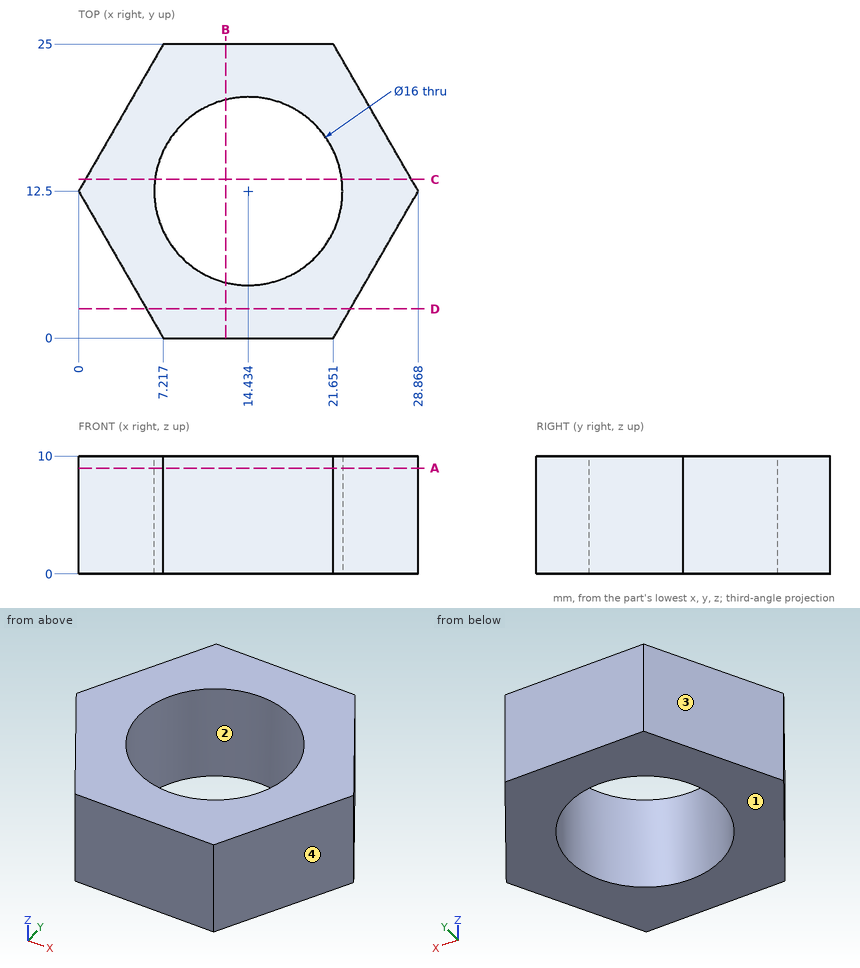
Here's the drawing with two shaded views (mm, measured from the low corner). I have some questions. Coordinates: 2 decimals unless noted, no trailing zeros. Order: outer loops, then holes, each group sorted by start corner. A loop starts at its lowest first (then second) coordinate and runs counter-clockwise, first axis right, second up.
Item 1: If we section it at D-D, the plane y = 2.5: List the corners of the cut face in (x, z) for me, then the cut area to 3 significant figures.
Response values:
outline: (5.77, 0) - (23.09, 0) - (23.09, 10) - (5.77, 10) - close
area: 173 mm2
Item 2: I'm going to push flat-ended pins straight in: pin 1 Ø1 at (x, z) = (6, 5.5) entering from -Y; pin 2 Ø1 at (x, z) = (4.5, 6) entering from +Y; pin 3 Ø1 at (x, z) = (6.5, 2) entering from -Y (1 decimal). Where does each tip first touch, or does it pass through?
Response values:
pin 1: stops at y = 1.24
pin 2: stops at y = 21.16
pin 3: stops at y = 0.4
Item 3: If we section it at A-A, the plane z = 9: List the corners of the cut face in (x, y) for me, then the cut area to 3 significant figures.
Response values:
outline: (0, 12.5) - (7.22, 0) - (21.65, 0) - (28.87, 12.5) - (21.65, 25) - (7.22, 25) - close; hole circle Ø16 at (14.43, 12.5)
area: 340 mm2
Item 4: Thinking about a two-plate mould opening in X: for the marked faces 1, 2, 3 and 4, which applies, pulls with the +X half, pulls with the -X half, needs draft (parallel to the pull), parting line crosses it, or undercut?
Response values:
face 1: needs draft
face 2: undercut
face 3: pulls with the -X half
face 4: pulls with the +X half
Item 5: If we section it at C-C, the plane y = 13.5: List the corners of the cut face in (x, z) for me, then the cut area to 3 significant figures.
Response values:
outline: (0.58, 0) - (6.5, 0) - (6.5, 10) - (0.58, 10) - close; (22.37, 0) - (28.29, 0) - (28.29, 10) - (22.37, 10) - close
area: 118 mm2
Item 6: If we section it at B-B, the plane x = 12.5: List the corners of the cut face in (y, z) for me.
Response values:
outline: (0, 0) - (4.74, 0) - (4.74, 10) - (0, 10) - close; (20.26, 0) - (25, 0) - (25, 10) - (20.26, 10) - close
Item 7: I need wall thicknesses on probe 1 along Y at (x, z) = (10, 3.25); probe 2 along X at (y, z) = (19.5, 5.5) (1 decimal); probe 3 along Y at (x, z) = (7.5, 1.25). Which ranges of each line are inside material? Lowest first, please.
Response values:
probe 1: y = 0 to 5.84, 19.16 to 25
probe 2: x = 4 to 10.6, 18.3 to 24.8
probe 3: y = 0 to 8.51, 16.49 to 25
